The listing builds one solid part. Answer for the finished solid, in the listing's coordinates (mm). A direction names the side the tool comes from. Round coordinates to 2 decimals unless told otherwise and drop trailing zeros. Order: outer loops, then holes, each group sorted by start corner. A loop starts at its lowest first (then second) coordinate and runs counter-clockwise, first axis right, second up. Notation, with made-up numbers: (57, -39.75) -> (75, -39.75) arc R6 ccw to (75, -31.75) -> close; hole circle Ø6 at (77, 69.25). An arc over 180 degrees is marked (long way). Return JSON: item names as keys, results as strings. Group by question number.
(1) Which of the six approach directions +Z, -Z, +X, -X, +Y, -Y give full straight-line access (tool end or side, diameter ignored) to faces 1 (the face through (179, -25, 0.4)), 2 (the face through (107.496, 0.33, 0.084)), 3 (the face through (253.9, -25.4, -0.4))?
(2) Determine the mould class of faces 4 (the face through (-4, -37.5, 0)), 5 (the face through (-257.5, -1, 0)), 6 (the face through (257.5, -1, 0)), 7 (the face through (186.995, -22.258, -2.845)) for opening direction X: +X half, -X half, draft (parallel to the pull), parting line (faces both ways), or undercut.
(3) The part is cut by section A-A (x = 80). Determine the outline of the cut face in (y, z), plus the area to 3 significant figures.
(4) Each of these flat-tipped pins is pushed along its axis until it touches: pin 1 (3 mm diameter, centred on x = 197.5, z = 0, fed in from -Y); pin 2 (4.5 mm diameter, centred on x = -197.5, z = 0, fed in from -Y); pin 3 (2.5 mm diameter, centred on x = 72, z = -0.5, fed in from +Y). Where does it stop, or does it pass through?
(5) Consider line 1 (Y direction, x = 141.5, z = -3.25); line 2 (Y direction, x = 221.5, z = 2.25); line 3 (X direction, y = 28, z = 3). Determine where each line is inside the solid, lowest interval first. Write a range as [from, to].
from build123d import *

# Parameters (mm, degrees)
SKETCH1_W                                           = 515
SKETCH1_H                                           = 75
BOSS_EXTRUDE1_DEPTH                                 = 6
M6_TAPPED_HOLE1_D                                   = 5
M6_TAPPED_HOLE1_DEPTH                               = 17
BLIND_PIN_HOLE2_D                                   = 8
CBORE_FOR_M6_HEX_SOCKET_HEAD_CAP_SCREW1_D           = 6.2
CBORE_FOR_M6_HEX_SOCKET_HEAD_CAP_SCREW1_CBORE_D     = 11
CBORE_FOR_M6_HEX_SOCKET_HEAD_CAP_SCREW1_CBORE_DEPTH = 6.4
M6_TAPPED_HOLE2_D                                   = 5
M6_TAPPED_HOLE3_D                                   = 5
M6_TAPPED_HOLE3_DEPTH                               = 12
M6_TAPPED_HOLE3_TIP                                 = 1.502151548
MM_2_D                                              = 5
MM_2_DEPTH                                          = 11
MM_2_TIP                                            = 1.502151548
CBORE_FOR_M6_HEX_SOCKET_HEAD_CAP_SCREW2_D           = 6.6
CBORE_FOR_M6_HEX_SOCKET_HEAD_CAP_SCREW2_CBORE_D     = 11
CBORE_FOR_M6_HEX_SOCKET_HEAD_CAP_SCREW2_CBORE_DEPTH = 6.4
CUT_EXTRUDE1_DEPTH                                  = 261.492802204
CHAMFER1_SIZE                                       = 1


with BuildPart() as part:
    # Sketch1 → Boss-Extrude1 (new, symmetric)
    with BuildSketch(Plane.XY):
        Rectangle(SKETCH1_W, SKETCH1_H)
    extrude(amount=BOSS_EXTRUDE1_DEPTH, both=True)

    # M6 Tapped Hole1
    with Locations(Plane(origin=(0, 37.5, 0), x_dir=(1, 0, 0), z_dir=(0, 1, 0))):
        with Locations((72, 0), (97, 0)):
            Hole(M6_TAPPED_HOLE1_D / 2, depth=M6_TAPPED_HOLE1_DEPTH)

    # Blind pin hole2 (through all)
    with Locations(Plane(origin=(0, 0, -6), x_dir=(-1, 0, 0), z_dir=(0, 0, -1))):
        with Locations((-141.5, 27.5), (-141.5, -17.5)):
            Hole(BLIND_PIN_HOLE2_D / 2)

    # CBORE for M6 Hex Socket Head Cap Screw1 (through all)
    with Locations(Plane.XY.offset(6)):
        with Locations((151.5, 23), (151.5, -23), (251.5, 23), (251.5, -23)):
            CounterBoreHole(CBORE_FOR_M6_HEX_SOCKET_HEAD_CAP_SCREW1_D / 2, CBORE_FOR_M6_HEX_SOCKET_HEAD_CAP_SCREW1_CBORE_D / 2, CBORE_FOR_M6_HEX_SOCKET_HEAD_CAP_SCREW1_CBORE_DEPTH)

    # M6 Tapped Hole2 (through all)
    with Locations(Plane.XY.offset(6)):
        with Locations((116.0005, 3.6), (130.0005, 3.6), (116.0005, -19.4), (130.0005, -19.4)):
            Hole(M6_TAPPED_HOLE2_D / 2)

    # M6 Tapped Hole3
    with Locations(Plane(origin=(0, -37.5, 0), x_dir=(-1, 0, 0), z_dir=(0, -1, 0))):
        with Locations((237.5, 0), (142.5, 0), (47.5, 0), (-47.5, 0), (-142.5, 0), (-237.5, 0)):
            Hole(M6_TAPPED_HOLE3_D / 2, depth=M6_TAPPED_HOLE3_DEPTH)
            with Locations((0, 0, -(M6_TAPPED_HOLE3_DEPTH + M6_TAPPED_HOLE3_TIP / 2))):  # 118° drill point
                Cone(0, M6_TAPPED_HOLE3_D / 2, M6_TAPPED_HOLE3_TIP, mode=Mode.SUBTRACT)

    # 大小mm 暗销孔2
    with Locations(Plane(origin=(0, -37.5, 0), x_dir=(-1, 0, 0), z_dir=(0, -1, 0))):
        with Locations((-197.5, 0), (197.5, 0)):
            Hole(MM_2_D / 2, depth=MM_2_DEPTH)
            with Locations((0, 0, -(MM_2_DEPTH + MM_2_TIP / 2))):  # 118° drill point
                Cone(0, MM_2_D / 2, MM_2_TIP, mode=Mode.SUBTRACT)

    # CBORE for M6 Hex Socket Head Cap Screw2 (through all)
    with Locations(Plane(origin=(0, 0, -6), x_dir=(-1, 0, 0), z_dir=(0, 0, -1))):
        with Locations((-221.5, 27.5), (-181.5, 27.5), (-181.5, -22.5), (-221.5, -22.5)):
            CounterBoreHole(CBORE_FOR_M6_HEX_SOCKET_HEAD_CAP_SCREW2_D / 2, CBORE_FOR_M6_HEX_SOCKET_HEAD_CAP_SCREW2_CBORE_D / 2, CBORE_FOR_M6_HEX_SOCKET_HEAD_CAP_SCREW2_CBORE_DEPTH)

    # Sketch18 → Cut-Extrude1 (cut, through all)
    with BuildSketch(Plane.XY.offset(6)):
        with BuildLine():
            Line((-227.5, 15), (-107.5, 15))
            ThreePointArc((-107.5, 15), (-92.5, 0), (-107.5, -15))
            Line((-107.5, -15), (-227.5, -15))
            ThreePointArc((-227.5, -15), (-242.5, 0), (-227.5, 15))
        make_face()
        with BuildLine():
            Line((-27.5, 15), (92.5, 15))
            ThreePointArc((92.5, 15), (107.5, 0), (92.5, -15))
            Line((92.5, -15), (-27.5, -15))
            ThreePointArc((-27.5, -15), (-42.5, 0), (-27.5, 15))
        make_face()
    extrude(amount=-CUT_EXTRUDE1_DEPTH, mode=Mode.SUBTRACT)

    # Chamfer1
    chamfer1_edges = [part.edges().sort_by_distance(p)[0] for p in [
        (257.5, -37.5, 0),
        (-257.5, -37.5, 0),
        (-257.5, 37.5, 0),
        (257.5, 37.5, 0),
    ]]
    chamfer(chamfer1_edges, length=CHAMFER1_SIZE)


solid = part.part
Answer below:
{
 "1": {"face 1": "-Z", "face 2": "+Z, -Z", "face 3": "+Z"},
 "2": {"face 4": "draft", "face 5": "-X half", "face 6": "+X half", "face 7": "undercut"},
 "3": {"outline": "(-37.5, -6) -> (-15, -6) -> (-15, 6) -> (-37.5, 6) -> close; (15, -6) -> (37.5, -6) -> (37.5, 6) -> (15, 6) -> close", "area": "540 mm²"},
 "4": {"pin 1": "stops at y = -25.9", "pin 2": "stops at y = -26.35", "pin 3": "stops at y = 20.5"},
 "5": {"line 1": "y = [-37.5, -21.5], [-13.5, 23.5], [31.5, 37.5]", "line 2": "y = [-37.5, -25.8], [-19.2, 24.2], [30.8, 37.5]", "line 3": "x = [-257.5, 137.53], [145.47, 149.21], [153.79, 178.24], [184.76, 218.24], [224.76, 249.21], [253.79, 257.5]"}
}
